```python
from build123d import *

# Parameters (mm, degrees)
BOSS_EXTRUDE1_DEPTH          = 113.3
SKETCH2_R                    = 6
CUT_EXTRUDE1_DEPTH           = 110
M8_TAPPED_HOLE_1_D           = 6.8
M8_TAPPED_HOLE_1_DEPTH       = 17
M8_TAPPED_HOLE_1_CSINK_D     = 8.05
M8_TAPPED_HOLE_1_CSINK_ANGLE = 90
M8_TAPPED_HOLE_1_TIP         = 2.042926105


with BuildPart() as part:
    # Sketch1 → Boss-Extrude1 (new body)
    with BuildSketch(Plane.XY):
        Polygon((-113, 41), (-87, 41), (-85, 39), (-85, 28), (-87, 26), (-113, 26), (-115, 28), (-115, 39), align=None)
    extrude(amount=BOSS_EXTRUDE1_DEPTH)

    # Sketch2 → Cut-Extrude1 (cut)
    with BuildSketch(Plane(origin=(0, 26, 0), x_dir=(-1, 0, 0), z_dir=(0, -1, 0))):
        with Locations(Location((100, -91.3, 0), (0, 0, 90))):
            Circle(SKETCH2_R)
    extrude(amount=-CUT_EXTRUDE1_DEPTH, mode=Mode.SUBTRACT)

    # M8 Tapped Hole 1
    with Locations(Plane(origin=(0, 0, 0), x_dir=(-1, 0, 0), z_dir=(0, 0, -1))):
        with Locations((100, 33.5)):
            CounterSinkHole(M8_TAPPED_HOLE_1_D / 2, M8_TAPPED_HOLE_1_CSINK_D / 2, depth=M8_TAPPED_HOLE_1_DEPTH, counter_sink_angle=M8_TAPPED_HOLE_1_CSINK_ANGLE)
            with Locations((0, 0, -(M8_TAPPED_HOLE_1_DEPTH + M8_TAPPED_HOLE_1_TIP / 2))):  # 118° drill point
                Cone(0, M8_TAPPED_HOLE_1_D / 2, M8_TAPPED_HOLE_1_TIP, mode=Mode.SUBTRACT)


solid = part.part
```
Read the model definition and answer for the solid it produces. Units are mm, in the model's axes. A direction names the side the tool comes from. Round coordinates to 2 decimals unless told otherwise and drop trailing zeros. Write each loop counter-clockwise with the first axis right and the second up, starting at its lowest first coordinate (ties: lowest second). Pieces come first, ordered by that corner, then holes. Notation, with made-up numbers: M 78,14.5 L 88,14.5 A24 cw 88,48.5 Z; hole C 9,-30 d11. An arc over 180 degrees is marked long. One line per item, written item: value.
Q1. Which of the six approach directions +Z, -Z, +X, -X, +Y, -Y give full straight-line access (tool end or side, diameter ignored) to faces 1 (the flat face through (-100, 26, 56)), 2 (the cylindrical face through (-103.4, 33.6, 8.9))?
Data:
face 1: +Z, -Z, +X, -X, -Y
face 2: -Z
Q2. For a pull along Y with two mould halves and no side action, classify faces 3 (the conical face through (-99.872, 32.924, 18.688)), 4 (the flat face through (-114, 27, 56)), 5 (the flat face through (-85, 34, 56)) as +Y half, -Y half, draft (parallel to the pull), parting line (faces both ways), or undercut.
Data:
face 3: undercut
face 4: -Y half
face 5: draft
Q3. Find section A-A on z = 91.3. Write down the section's boundary in (x, y).
Data:
outline: M -115,28 L -113,26 L -106,26 L -106,41 L -113,41 L -115,39 Z; M -94,26 L -87,26 L -85,28 L -85,39 L -87,41 L -94,41 Z
Q4. Find section B-B on z = 63. Write down the section's boundary in (x, y), plus the area to 3 significant figures.
Data:
outline: M -115,28 L -113,26 L -87,26 L -85,28 L -85,39 L -87,41 L -113,41 L -115,39 Z
area: 442 mm2
Q5. Flat-ended cylindrical pins translate along their axes: pin 1 Ø3 at (x, z) = (-103, 93.5) entering from -Y; pin 2 Ø6 at (x, y) = (-100, 33.5) entering from -Z. Find the tip coordinate at first contact, or state that the pin passes through.
Data:
pin 1: through
pin 2: z = 17.24
Q6. Straight lines are drawn through the part: line 1 (Y direction, x = -100, z = 12); line 2 (X direction, y = 36.75, z = 91.3); line 3 (Z direction, x = -102.25, y = 27.75). For each, find the intervals that lie inside material, in ascending order. Write a range as [from, to].
Data:
line 1: [26, 30.1], [36.9, 41]
line 2: [-115, -106], [-94, -85]
line 3: [0, 85.74], [96.86, 113.3]
